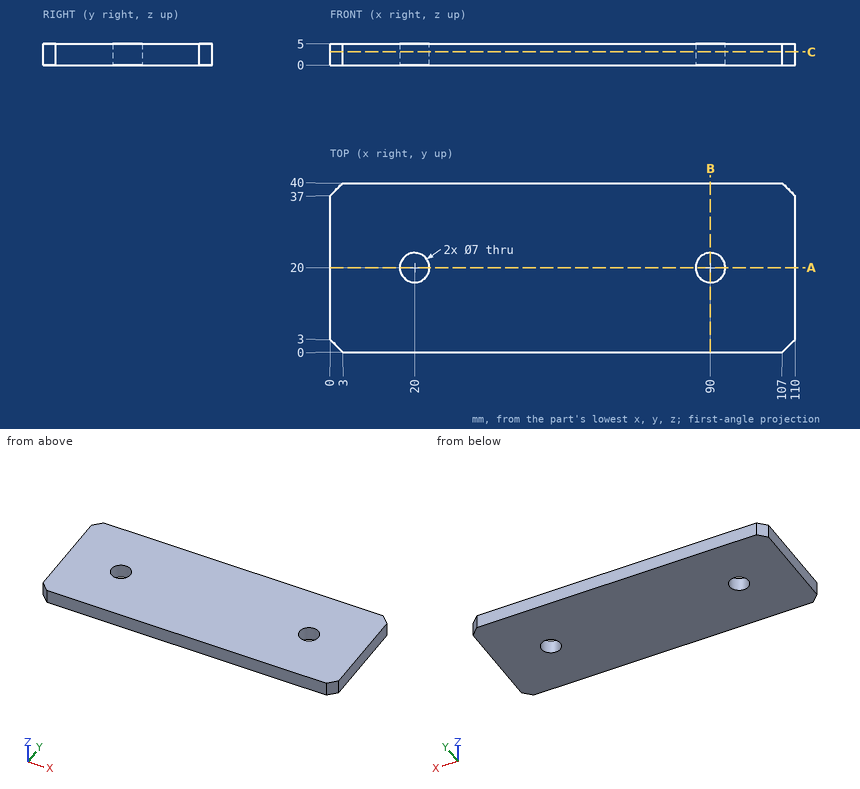
Drawing for the job (mm, zero at the part's lowest x, y, z). Coordinates: 2 decimals unless noted, no trailing zeros. Order: outer loops, then holes, each group sorted by start corner. A loop starts at its lowest first (then second) coordinate and runs counter-clockwise, first axis right, second up. Notation, with made-up numbers: (9.5, 79.25) -> (43.5, 79.25) arc R26 cw to (43.5, 102.25) -> close; hole circle Ø4 at (-32.5, 70.25). An arc over 180 degrees is marked (long way). One line per item, written item: value.
(1) Slice it at A-A, the plane y = 20. List the corners of the cut face in (x, z).
Checked values:
outline: (0, 0) -> (16.5, 0) -> (16.5, 5) -> (0, 5) -> close; (23.5, 0) -> (86.5, 0) -> (86.5, 5) -> (23.5, 5) -> close; (93.5, 0) -> (110, 0) -> (110, 5) -> (93.5, 5) -> close
(2) Drop a flat-ended pin along its axis: pin 1 Ø3 at (x, y) = (21, 22.5) entering from -Z. Give the stop position or say it passes through.
Checked values:
pin 1: z = 0
(3) Slice it at B-B, the plane x = 90. List the corners of the cut face in (y, z).
Checked values:
outline: (0, 0) -> (16.5, 0) -> (16.5, 5) -> (0, 5) -> close; (23.5, 0) -> (40, 0) -> (40, 5) -> (23.5, 5) -> close
(4) Probe line 1 (Y direction, x = 90, z = 2.35); line 2 (Y direction, x = 18, z = 2.5). List the from-to ranges inside material, lowest first. Write a range as [from, to].
Checked values:
line 1: [0, 16.5], [23.5, 40]
line 2: [0, 17.13], [22.87, 40]
(5) Slice it at C-C, the plane z = 3.15. List the corners of the cut face in (x, y), plus the area to 3 significant figures.
Checked values:
outline: (0, 3) -> (3, 0) -> (107, 0) -> (110, 3) -> (110, 37) -> (107, 40) -> (3, 40) -> (0, 37) -> close; hole circle Ø7 at (20, 20); hole circle Ø7 at (90, 20)
area: 4,310 mm2
